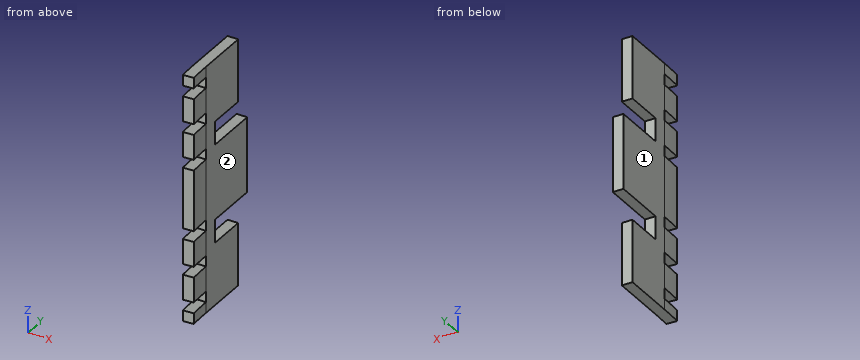
```python
from build123d import *

# Parameters (mm, degrees)
BOSS_EXTRUDE1_DEPTH = 69
SKETCH5_W           = 6
SKETCH5_H           = 28.749782116
CUT_EXTRUDE5_DEPTH  = 250.384613791
CUT_EXTRUDE1_DEPTH  = 80.350082519


with BuildPart() as part:
    # Sketch1 → Boss-Extrude1 (new, symmetric)
    with BuildSketch(Plane.XY):
        with BuildLine():
            Line((-236.175884969, -12.377453651), (-230.184107761, -12.063437914))
            ThreePointArc((-230.184107761, -12.063437914), (-230.421013407, -6.033786585), (-230.5, 0))
            Line((-230.5, 0), (-230.5, 38.722546349))
            Line((-230.5, 38.722546349), (-236.5, 38.722546349))
            Line((-236.5, 38.722546349), (-236.5, 0))
            ThreePointArc((-236.5, 0), (-236.418957357, -6.190848275), (-236.175884969, -12.377453651))
        make_face()
    extrude(amount=BOSS_EXTRUDE1_DEPTH, both=True)

    # Sketch5 → Cut-Extrude5 (cut, through all)
    with BuildSketch(Plane(origin=(0, 0, 0), x_dir=(0, 0, -1), z_dir=(1, 0, 0))):
        with Locations((-60, -14.374891058)):
            Rectangle(SKETCH5_W, SKETCH5_H)
        with Locations((-40, -14.374891058)):
            Rectangle(SKETCH5_W, SKETCH5_H)
        with Locations((-20, -14.374891058)):
            Rectangle(SKETCH5_W, SKETCH5_H)
        with Locations((20, -14.374891058)):
            Rectangle(SKETCH5_W, SKETCH5_H)
        with Locations((40, -14.374891058)):
            Rectangle(SKETCH5_W, SKETCH5_H)
        with Locations((60, -14.374891058)):
            Rectangle(SKETCH5_W, SKETCH5_H)
    extrude(amount=-CUT_EXTRUDE5_DEPTH, mode=Mode.SUBTRACT)

    # Sketch3 → Cut-Extrude1 (cut, through all)
    with BuildSketch(Plane(origin=(-230.5, 0, 0), x_dir=(0, 0, -1), z_dir=(1, 0, 0))):
        Polygon((-69, 30.222546349), (-34, 30.222546349), (-34, 8.522546349), (-21, 8.522546349), (-21, 38.722546349), (-69, 38.722546349), align=None)
        Polygon((21, 8.522546349), (21, 38.722546349), (69, 38.722546349), (69, 30.222546349), (34, 30.222546349), (34, 8.522546349), align=None)
    extrude(amount=-CUT_EXTRUDE1_DEPTH, mode=Mode.SUBTRACT)


solid = part.part
```
Here's how the part is built. I have some questions about the finished solid (model axes, mm). Face numbers are marked on the shaded views. A direction names the side the tool comes from. Coordinates: 2 decimals unless noted, no trailing zeros. Order: outer loops, then holes, each group sorted by start corner. A loop starts at its lowest first (then second) coordinate and runs counter-clockwise, first axis right, second up. Notation, with made-up numbers: (26.5, 14.5) - (57.5, 14.5) arc R16 cw to (57.5, 20.5) - close; hole circle Ø9 at (4, 15). An arc over 180 degrees is marked (long way). One line per question, with ' | ' between items. Start each with the question number.
1. If we section it at D-D (z = 30): Write out the boundary of the cut face in (x, y).
2. Please list where these lines run through material, in increasing order: line 1 along Z through (x, y) = (-230.75, 25); line 2 along Y through (x, z) = (-230.75, 39.5); line 3 along X through (y, z) = (9, 11). Write a range as [from, to].
3. I'm going to push flat-ended pins straight in: pin 1 Ø12 at (y, z) = (22.5, 27.5) entering from -X; pin 2 Ø1.8 at (x, z) = (-233.5, 19) entering from -Y; pin 3 Ø1.8 at (x, z) = (-235, 26) entering from +Y; pin 4 Ø1.8 at (x, z) = (-232, -45) entering from +Y. Where does each tip first touch, or does it pass through?
4. If we section it at C-C (z = -10.5): Write out the boundary of the cut face in (x, y).
5. If we section it at A-A (y = 18): Write out the boundary of the cut face in (x, z).
6. Which directions (+Z, -Z, +X, -X, +Y, -Y) give clear straight access to the entire face, cutting with the end or side of a thin tool? Please do the marked faces 1 and 2.
7. If we section it at B-B (y = -6): Write out the boundary of the cut face in (x, z).
Model answer:
1) outline: (-236.5, 0) arc R236.5 ccw to (-236.18, -12.38) - (-230.18, -12.06) arc R230.5 cw to (-230.5, 0) - (-230.5, 8.52) - (-236.5, 8.52) - close
2) line 1: z = [-69, -34], [-21, 21], [34, 69] | line 2: y = [0, 30.22] | line 3: x = [-236.5, -230.5]
3) pin 1: passes through | pin 2: stops at y = 0 | pin 3: stops at y = 8.52 | pin 4: stops at y = 30.22
4) outline: (-236.5, 0) arc R236.5 ccw to (-236.18, -12.38) - (-230.18, -12.06) arc R230.5 cw to (-230.5, 0) - (-230.5, 38.72) - (-236.5, 38.72) - close
5) outline: (-236.5, -69) - (-230.5, -69) - (-230.5, -34) - (-236.5, -34) - close; (-236.5, -21) - (-230.5, -21) - (-230.5, 21) - (-236.5, 21) - close; (-236.5, 34) - (-230.5, 34) - (-230.5, 69) - (-236.5, 69) - close
6) face 1: +Z, -Z, -X, +Y, -Y | face 2: +Z, -Z, +X, +Y
7) outline: (-236.42, -69) - (-230.42, -69) - (-230.42, -63) - (-236.42, -63) - close; (-236.42, -57) - (-230.42, -57) - (-230.42, -43) - (-236.42, -43) - close; (-236.42, -37) - (-230.42, -37) - (-230.42, -23) - (-236.42, -23) - close; (-236.42, -17) - (-230.42, -17) - (-230.42, 17) - (-236.42, 17) - close; (-236.42, 23) - (-230.42, 23) - (-230.42, 37) - (-236.42, 37) - close; (-236.42, 43) - (-230.42, 43) - (-230.42, 57) - (-236.42, 57) - close; (-236.42, 63) - (-230.42, 63) - (-230.42, 69) - (-236.42, 69) - close
